Can you work these out from the model? Positions are in its coordinate system, mm. A direction names the side the tool comes from. Round coordinates to 2 decimals unless told otherwise and drop trailing zeros. Order: outer loops, then holes, each group sorted by start corner. A loop starts at its lowest first (then second) coordinate and runs counter-clockwise, first axis right, second up. Notation, with made-up numbers: (-11, 63) -> (44, 63) arc R14 ccw to (44, 76) -> close; hole circle Ø4 at (58.5, 48). An arc over 180 degrees is marked (long way). Use a Markdown table: item, result. Add a question column.
Q1. If we section it at A-A on x = 42: List the corners of the cut face in (y, z) for me.
Q2. I'm going to push flat-ended pins straight in: pin 1 Ø2 at (y, z) = (85, -10.5) entering from -X; pin 2 Ø1.5 at (y, z) = (154, 10) entering from +X. Where does each tip first touch, or does it pass through?
Q3. We'd pull the mould along Z, two halves only. Please class faces 3 (the face through (31, 0, -14)), 4 (the face through (36, 89, -11)), 5 (the face through (31, 89, 21)), 6 (the face through (31, 89, -21)): +Z half, -Z half, draft (parallel to the pull), parting line (faces both ways), or undercut.
Q4. For faces 1 (the face through (10, 89, 0)), 2 (the face through (46.623, 27.252, -15.93)), which set-ups out of +Z, -Z, +X, -X, +Y, -Y let a thin tool reach every point of the face, with its end or its side?
Q5. If we section it at B-B on y = 160: List the corners of the cut face in (x, z) for me.
Q6. If we section it at C-C on x = 19: List the corners of the cut face in (y, z) for me.
Q7. I need wall thicknesses on line 1 along Y through (x, z) = (42, -18); line 2 along Z through (x, y) = (43, 74.5); line 3 along X through (y, z) = (13.5, -4). Which ranges of each line are inside material? Lowest first, please. Write a range as [from, to].
Q8. If we section it at D-D on z = -15: List the corners of the cut face in (x, y) for me, plus the area to 3 significant figures.
```python
from build123d import *

# Parameters (mm, degrees)
EXTRUDE_1_DEPTH     = 180
SKETCH_2_R          = 8.6
CUT_EXTRUDE_1_DEPTH = 195.956405383


with BuildPart() as part:
    # 草图1 → 凸台-拉伸1 (new body)
    with BuildSketch(Plane(origin=(0, 0, 0), x_dir=(1, 0, 0), z_dir=(0, 1, 0))):
        Polygon((62, 11), (10, 11), (10, -11), (62, -11), (62, -21), (0, -21), (0, 21), (62, 21), align=None)
    extrude(amount=EXTRUDE_1_DEPTH)

    # 草图2 → 切除-拉伸1 (cut, through all)
    with BuildSketch(Plane.XY.offset(21)):
        with Locations((42, 160)):
            Circle(SKETCH_2_R)
        with Locations((42, 20)):
            Circle(SKETCH_2_R)
    extrude(amount=-CUT_EXTRUDE_1_DEPTH, mode=Mode.SUBTRACT)


solid = part.part
```
Answer below:
| question | item | result |
|---|---|---|
| 1 | outline | (0, -21) -> (11.4, -21) -> (11.4, -11) -> (0, -11) -> close; (0, 11) -> (11.4, 11) -> (11.4, 21) -> (0, 21) -> close; (28.6, -21) -> (151.4, -21) -> (151.4, -11) -> (28.6, -11) -> close; (28.6, 11) -> (151.4, 11) -> (151.4, 21) -> (28.6, 21) -> close; (168.6, -21) -> (180, -21) -> (180, -11) -> (168.6, -11) -> close; (168.6, 11) -> (180, 11) -> (180, 21) -> (168.6, 21) -> close |
| 2 | pin 1 | x = 0 |
| 2 | pin 2 | x = 10 |
| 3 | face 3 | draft |
| 3 | face 4 | undercut |
| 3 | face 5 | +Z half |
| 3 | face 6 | -Z half |
| 4 | face 1 | +X, +Y, -Y |
| 4 | face 2 | +Z, -Z |
| 5 | outline | (0, -21) -> (33.4, -21) -> (33.4, -11) -> (10, -11) -> (10, 11) -> (33.4, 11) -> (33.4, 21) -> (0, 21) -> close; (50.6, -21) -> (62, -21) -> (62, -11) -> (50.6, -11) -> close; (50.6, 11) -> (62, 11) -> (62, 21) -> (50.6, 21) -> close |
| 6 | outline | (0, -21) -> (180, -21) -> (180, -11) -> (0, -11) -> close; (0, 11) -> (180, 11) -> (180, 21) -> (0, 21) -> close |
| 7 | line 1 | [0, 11.4], [28.6, 151.4], [168.6, 180] |
| 7 | line 2 | [-21, -11], [11, 21] |
| 7 | line 3 | [0, 10] |
| 8 | outline | (0, 0) -> (62, 0) -> (62, 180) -> (0, 180) -> close; hole circle Ø17.2 at (42, 20); hole circle Ø17.2 at (42, 160) |
| 8 | area | 10,700 mm² |
